Part print with two shaded views. Sizes in mm from the minimum x, y, z corner. A direction names the side the tool comes from. Give positions to 0.01 mm unless a question says otherwise; leave off trailing zeros. Order: outer loops, then holes, each group sorted by start corner. A loop starts at its lowest first (then second) coordinate and runs counter-clockwise, first axis right, second up. Notation, with made-up numbers: (45, 30) -> (64, 30) arc R19 ccw to (64, 39) -> close; hole circle Ø6 at (-26, 34.25). An arc over 180 degrees is marked (long way). Answer as CSV lines item,"result".
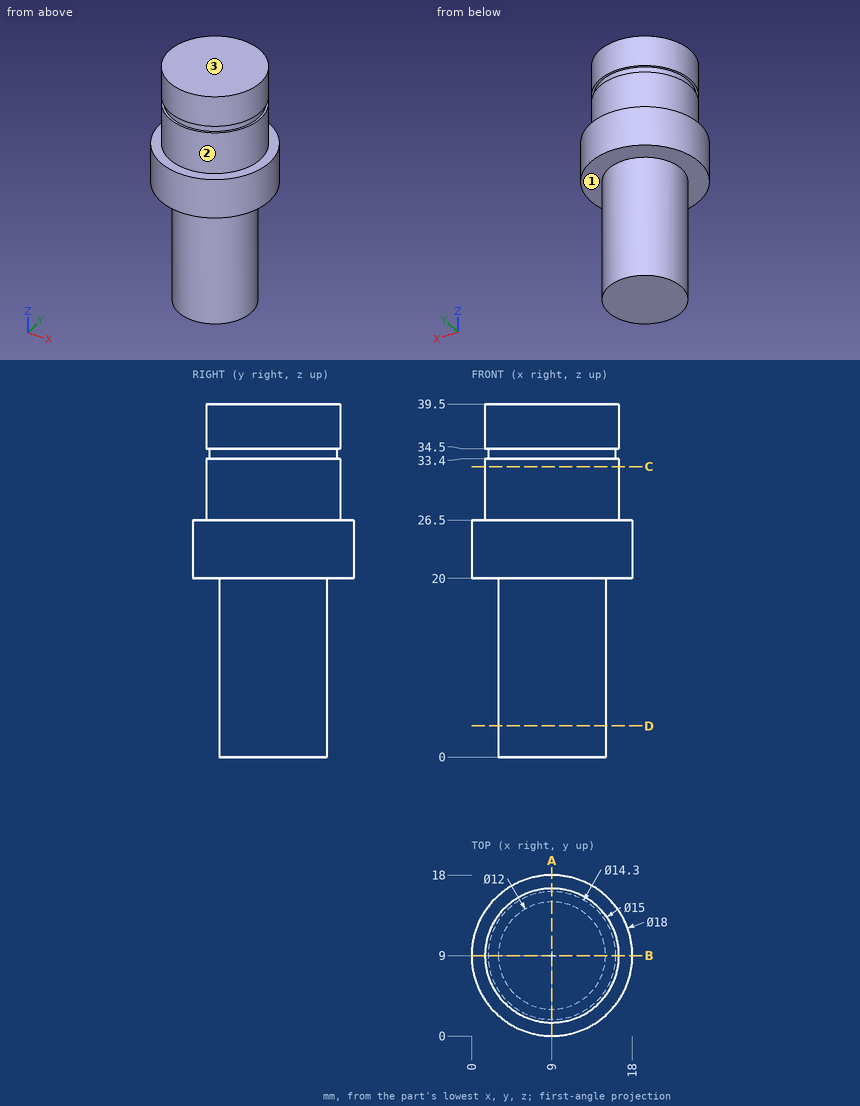
1) Band-saw the part on A-A, the plane x = 9. Write the cut outline in (y, z), then the cut area to 3 significant figures.
Data:
outline,"(0, 20) -> (3, 20) -> (3, 0) -> (15, 0) -> (15, 20) -> (18, 20) -> (18, 26.5) -> (16.5, 26.5) -> (16.5, 33.4) -> (16.15, 33.4) -> (16.15, 34.5) -> (16.5, 34.5) -> (16.5, 39.5) -> (1.5, 39.5) -> (1.5, 34.5) -> (1.85, 34.5) -> (1.85, 33.4) -> (1.5, 33.4) -> (1.5, 26.5) -> (0, 26.5) -> close"
area,"551 mm2"
2) Pin check, flat tips, straight feed: P1, Ø4, axis at x = 9.5, z = 11, coming from the -Y side; P2, Ø6, axis at y = 9, z = 6, coming from the -X side; P3, Ø5, axis at y = 13.5, z = 16, coming from the +X side. Stop position of each tip, or through.
Data:
P1,"stops at y = 3"
P2,"stops at x = 3"
P3,"stops at x = 14.66"
3) Band-saw the part on D-D, the plane z = 3.5. Write the cut outline in (x, y).
Data:
outline,"circle Ø12 at (9, 9)"
4) Wall check: line 1 along Z through (x, y) = (15, 5.25); line 2 along X through (y, z) = (8.75, 4); line 3 along X through (y, z) = (12, 18). Give the ranges that are in metal, low to high. Write a range as [from, to].
Data:
line 1,"z = [20, 39.5]"
line 2,"x = [3.01, 14.99]"
line 3,"x = [3.8, 14.2]"
5) Which spindle directions (+Z, -Z, +X, -X, +Y, -Y) get a long thin tool onto all of the face, cutting with end or side? Do the marked faces 1, 2 and 3. Say none if no direction does.
Data:
face 1,"-Z"
face 2,"+Z"
face 3,"+Z, +X, -X, +Y, -Y"
6) Band-saw the part on C-C, the plane z = 32.5. Write the cut outline in (x, y).
Data:
outline,"circle Ø15 at (9, 9)"
